Source: CAD feature listing. Evaluate the final solid. Frame: model axes, mm. Coordinates: 2 decimals unless noted, no trailing zeros. Write each loop counter-clockwise with the first axis right and the second up, starting at its lowest first coordinate (ties: lowest second). Pieces come first, ordered by that corner, then holes. Notation, with made-up numbers: (22.5, -26) -> (32.5, -26) arc R11 cw to (32.5, -16) -> close; hole circle Ø6 at (-9.75, -6.5). An arc over 180 degrees is marked (long way). Write item = value, one per line.
from build123d import *

# Parameters (mm, degrees)
SKETCH1_R           = 6.5
SKETCH1_R_2         = 3
BOSS_EXTRUDE1_DEPTH = 5
CHAMFER1_SIZE       = 0.1


with BuildPart() as part:
    # Sketch1 → Boss-Extrude1 (new body)
    with BuildSketch(Plane.XY):
        Circle(SKETCH1_R)
        Circle(SKETCH1_R_2, mode=Mode.SUBTRACT)
    extrude(amount=BOSS_EXTRUDE1_DEPTH)

    # Chamfer1
    chamfer1_edges = [part.edges().sort_by_distance(p)[0] for p in [
        (-6.5, 0, 0),
        (-6.5, 0, 5),
        (-3, 0, 0),
        (-3, 0, 5),
    ]]
    chamfer(chamfer1_edges, length=CHAMFER1_SIZE)


solid = part.part
1) Cut plane A-A, the plane x = 0. Output: boundary loops of the cut face in (y, z).
Answer block:
outline = (-6.5, 0.1) -> (-6.4, 0) -> (-3.1, 0) -> (-3, 0.1) -> (-3, 4.9) -> (-3.1, 5) -> (-6.4, 5) -> (-6.5, 4.9) -> close; (3, 0.1) -> (3.1, 0) -> (6.4, 0) -> (6.5, 0.1) -> (6.5, 4.9) -> (6.4, 5) -> (3.1, 5) -> (3, 4.9) -> close
2) Cut plane C-C, the plane z = 1.95. Output: boundary loops of the cut face in (x, y), and give its area (3 significant figures).
Answer block:
outline = circle Ø13 at (0, 0); hole circle Ø6 at (0, 0)
area = 104 mm2
3) First-contact query: pin 1 Ø2 at (y, z) = (-4.5, 1.5) entering from -X. Flat tip, straight axial feed; report the tip coordinate or a pass-through.
Answer block:
pin_1 = -5.48
4) Pull-direction query (Y, two-part tool) for faces 1 (the cylindrical face through (-3, 0, 2)), 2 (the cylindrical face through (-5.158, -3.955, 2.466)), 3 (the flat face through (3, 2, 5)); classes: +Y half, -Y half, draft (parallel to the pull), parting line (faces both ways), or undercut.
Answer block:
face_1 = undercut
face_2 = parting line
face_3 = draft
5) Material intervals for probe 1 along Y at (x, z) = (0, 3.5); probe 2 along X at (y, z) = (-1, 1.8); probe 3 along X at (y, z) = (1.5, 3.05), sorted ascending. Write a range as [from, to].
Answer block:
probe_1 = [-6.5, -3], [3, 6.5]
probe_2 = [-6.42, -2.83], [2.83, 6.42]
probe_3 = [-6.32, -2.6], [2.6, 6.32]
